from build123d import *

# Parameters (mm, degrees)
SKETCH_2_R        = 7.94
EXTRUDE_1_DEPTH   = 7.875
EXTRUDE_1_2_DEPTH = 7.875
EXTRUDE_2_DEPTH   = 3.43
SKETCH_6_R        = 3.97
EXTRUDE_4_DEPTH   = 3.34
SCALE_1_SCALE     = 0.65


with BuildPart() as part:
    # Sketch 2 → Extrude 1 (new, symmetric)
    with BuildSketch(Plane.XY):
        with Locations((12.7, 0)):
            Circle(SKETCH_2_R)
    extrude(amount=EXTRUDE_1_DEPTH, both=True)



with BuildPart() as body_2:
    # Sketch 2 → Extrude 1 2 (new, symmetric)
    with BuildSketch(Plane.XY):
        with Locations((-12.7, 0)):
            Circle(SKETCH_2_R)
    extrude(amount=EXTRUDE_1_2_DEPTH, both=True)


with BuildPart() as part_1:
    add(part.part)

    add(body_2.part)  # Extrude 2 merges body 2
    # Sketch 3 → Extrude 2 (add)
    with BuildSketch(Plane.XY.offset(7.875)):
        with BuildLine():
            ThreePointArc((-10.428153415, 11.849174574), (-24.765, 0), (-10.428153415, -11.849174574))
            ThreePointArc((-10.428153415, -11.849174574), (0, -10.8585), (10.428153415, -11.849174574))
            ThreePointArc((10.428153415, -11.849174574), (24.765, 0), (10.428153415, 11.849174574))
            ThreePointArc((10.428153415, 11.849174574), (0, 10.8585), (-10.428153415, 11.849174574))
        make_face()
    extrude(amount=EXTRUDE_2_DEPTH)


with BuildPart() as body_2_2:
    # Sketch 6 → Extrude 4 (new body)
    with BuildSketch(Plane.XY.offset(11.305)):
        with BuildLine():
            ThreePointArc((32.154770058, -17.228648829), (48.987968132, -9.317166623), (38.048309834, 5.725173103))
            ThreePointArc((38.048309834, 5.725173103), (27.701405286, 7.358998688), (17.847242234, 10.911925695))
            ThreePointArc((17.847242234, 10.911925695), (1.014044161, 3.000443489), (11.953702459, -12.041896237))
            ThreePointArc((11.953702459, -12.041896237), (22.300607007, -13.675721822), (32.154770058, -17.228648829))
        make_face()
        with Locations((12.7, 0)):
            Circle(SKETCH_6_R, mode=Mode.SUBTRACT)
        with Locations((37.302012293, -6.316723134)):
            Circle(SKETCH_6_R, mode=Mode.SUBTRACT)
    extrude(amount=EXTRUDE_4_DEPTH)


with BuildPart() as body_2_2_1:
    # Scale 1: scaled about (0, 0, 0)
    add(body_2_2.part.scale(SCALE_1_SCALE))


solid = body_2_2_1.part
Verification items for the finished model (mm, model axes). Coordinates: 2 decimals unless noted, no trailing zeros. Order: outer loops, then holes, each group sorted by start corner. A loop starts at its lowest first (then second) coordinate and runs counter-clockwise, first axis right, second up. Notation, with made-up numbers: M -21.5,58.5 L 14.5,58.5 A14 cw 14.5,72.5 Z; hole C -4.75,85.25 d10. An arc over 180 degrees is marked long. One line per item, written item: value. Start each with the question number.
Item 1: Sectioned sample at C-C (y = 5.5). Enter the section's corners in (x, z), then the cut area to 3 significant figures.
Item 2: Sectioned sample at B-B (z = 8.65). Enter the section's corners in (x, y) (1 decimal).
Item 3: Sectioned sample at D-D (x = 4). Enter the section's corners in (y, z), then the cut area to 3 significant figures.
Item 4: Mould release check, pull along X, two halves, no side actions. Record for faces 1 (the cylindrical face through (10.716, 0.775, 8.419)), 2 (the flat face through (16, -2, 9.519)), 3 (the cylindrical face through (0.7, 2.1, 8.4)): released by +X, released by -X, zero draft, split by the parting line, or undercut.
Item 5: Scan lines: probe 1 along Y at (x, z) = (24.5, 9); probe 2 along Y at (x, z) = (7.5, 9.3); probe 3 along X at (y, z) = (-5.25, 8.1). Record each from-to range of solid material in increasing order.
Item 6: Gauge pin test, flat end, axial feed: pin 1 (3 mm diameter, centred on x = 8.255, y = 0, fed in from +Z). Record the tip position at first contact, or that the pin passes through.
Item 7: Sectioned sample at A-A (y = 1). Enter the section's corners in (x, z).
Conclusion:
1. outline: M 2.66,7.35 L 15.57,7.35 L 15.57,9.52 L 2.66,9.52 Z
1. area: 28.0 mm^2
2. outline: M 7.8,-7.8 A36 cw 20.9,-11.2 A7.8 ccw long 24.7,3.7 A36 cw 11.6,7.1 A7.8 ccw long Z; hole C 8.3,0 d5.2; hole C 24.2,-4.1 d5.2
3. outline: M -6.59,7.35 L 6.59,7.35 L 6.59,9.52 L -6.59,9.52 Z
3. area: 28.6 mm^2
4. face 1: undercut
4. face 2: zero draft
4. face 3: split by the parting line
5. probe 1: y = -11.94 to -6.67, -1.54 to 3.74
5. probe 2: y = -7.81 to -2.47, 2.47 to 7.81
5. probe 3: x = 2.43 to 21.93, 26.56 to 32
6. pin 1: passes through
7. outline: M 0.48,7.35 L 5.88,7.35 L 5.88,9.52 L 0.48,9.52 Z; M 10.63,7.35 L 30.2,7.35 L 30.2,9.52 L 10.63,9.52 Z
